Geometry check sheet. Reference: the model listing, model coordinates, mm. Face numbers are marked on the shaded views. A direction names the side the tool comes from. Give positions to 0.01 mm unless a question says otherwise; leave off trailing zeros. Loops run counter-clockwise (first coordinate to the right, second up) from the corner with the lowest first, then second, coordinate; pieces in that order, holes last. Notation, with made-up numbers: (65.25, 68.25) -> (124.25, 68.25) arc R19 ccw to (124.25, 85.25) -> close; hole circle Ø1 at (41, -15). An arc over 180 degrees is marked (long way). Answer as a JSON object with one key per item and string values.
from build123d import *

# Parameters (mm, degrees)
CHAMFER_1_SIZE           = 1
FILLET_1_R               = 2
CUT_EXTRUDE_1_DEPTH      = 99.642029582
CUT_EXTRUDE_1_DEPTH_BACK = 99.642029582
SKETCH_3_R               = 2.5


with BuildPart() as part:
    # 草图1 → 旋转1 (revolve)
    with BuildSketch(Plane.XY, mode=Mode.PRIVATE) as revolve_1_sk:
        with BuildLine():
            Line((0, 14.5), (13.774977314, 14.5))
            ThreePointArc((13.774977314, 14.5), (19.953843795, 1.357982993), (15.612494996, -12.5))
            Line((15.612494996, -12.5), (10.5, -12.5))
            Line((10.5, -12.5), (14.7, -39.5))
            Line((14.7, -39.5), (13.4, -69.5))
            Line((13.4, -69.5), (11.5, -69.5))
            Line((11.5, -69.5), (11.5, -94.5))
            Line((11.5, -94.5), (0, -94.5))
            Line((0, -94.5), (0, -12.5))
            Line((0, -12.5), (0, 14.5))
        make_face()
    revolve(revolve_1_sk.sketch.rotate(Axis((0, 41.043678396, 0), (0, -1, 0)), 90), axis=Axis((0, 41.043678396, 0), (0, -1, 0)))

    # 倒角1
    chamfer_1_edges = [part.edges().sort_by_distance(p)[0] for p in [
        (0, -94.5, -11.5),
    ]]
    chamfer(chamfer_1_edges, length=CHAMFER_1_SIZE)

    # 圆角1
    fillet_1_edges = [part.edges().sort_by_distance(p)[0] for p in [
        (0, -12.5, -10.5),
    ]]
    fillet(fillet_1_edges, radius=FILLET_1_R)

    # 草图3 → 切除-拉伸1 (cut, two sides: drawn at the far end of the back side and taken through both)
    with BuildSketch(Plane.XY.offset(-CUT_EXTRUDE_1_DEPTH_BACK)):
        with Locations((0, -88.5)):
            Circle(SKETCH_3_R)
    extrude(amount=CUT_EXTRUDE_1_DEPTH + CUT_EXTRUDE_1_DEPTH_BACK, mode=Mode.SUBTRACT)


solid = part.part
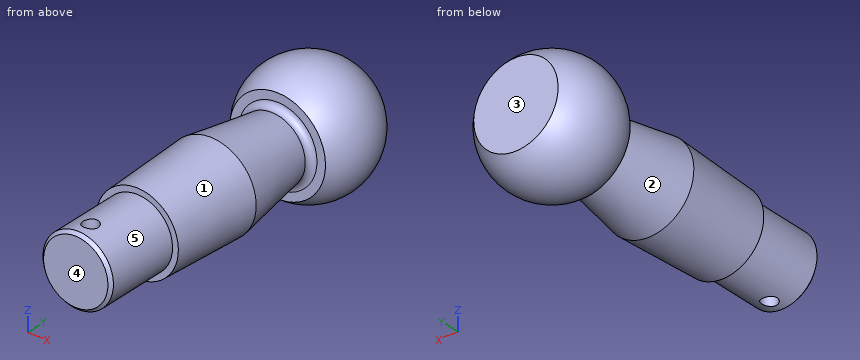
1) Section check B-B on z = 0. Record the cut outline in (x, y), plus the area to 3 significant figures.
Geometry check:
{"outline": "(-15.61, -12.5) -> (-12.84, -12.5) arc R2 cw to (-10.86, -14.81) -> (-14.7, -39.5) -> (-13.4, -69.5) -> (-11.5, -69.5) -> (-11.5, -93.5) -> (-10.5, -94.5) -> (10.5, -94.5) -> (11.5, -93.5) -> (11.5, -69.5) -> (13.4, -69.5) -> (14.7, -39.5) -> (10.86, -14.81) arc R2 cw to (12.84, -12.5) -> (15.61, -12.5) arc R20 ccw to (13.77, 14.5) -> (-13.77, 14.5) arc R20 ccw to start; hole circle Ø5 at (0, -88.5)", "area": "3,070 mm2"}
2) Tool access check on the marked faces 4 and 5. Record the directions out of +Z, -Z, +X, -X, +Y, -Y that give a thin tool (end or side, any length) a straight path to the whole face; none if there is none.
Geometry check:
{"face 4": "+Z, -Z, +X, -X, -Y", "face 5": "-Y"}
3) Section check A-A on x = 0. Record the cut outline in (y, z), plus the area to 3 significant figures.
Geometry check:
{"outline": "(-94.5, -10.5) -> (-93.5, -11.5) -> (-91, -11.5) -> (-91, 11.5) -> (-93.5, 11.5) -> (-94.5, 10.5) -> close; (-86, -11.5) -> (-69.5, -11.5) -> (-69.5, -13.4) -> (-39.5, -14.7) -> (-14.81, -10.86) arc R2 cw to (-12.5, -12.84) -> (-12.5, -15.61) arc R20 ccw to (14.5, -13.77) -> (14.5, 13.77) arc R20 ccw to (-12.5, 15.61) -> (-12.5, 12.84) arc R2 cw to (-14.81, 10.86) -> (-39.5, 14.7) -> (-69.5, 13.4) -> (-69.5, 11.5) -> (-86, 11.5) -> close", "area": "2,970 mm2"}
4) Draft check along Y on the marked faces 1, 2 and 3. Enter one of: pulls with the +Y half, pulls with the -Y half, needs draft (parallel to the pull), parting line crosses it, or undercut.
Geometry check:
{"face 1": "pulls with the -Y half", "face 2": "undercut", "face 3": "pulls with the +Y half"}
5) Section check D-D on y = 7. Record the cut outline in (x, z) (3 decimals), plus the area to 3 significant figures.
Geometry check:
{"outline": "circle Ø37.47 at (0, 0)", "area": "1,100 mm2"}
6) Section check C-C on y = -88.5. Record the cut outline in (x, z), plus the area to 3 significant figures.
Geometry check:
{"outline": "(-2.5, -11.22) -> (-2.5, 11.22) arc R11.5 ccw to start; (2.5, -11.22) arc R11.5 ccw to (2.5, 11.22) -> close", "area": "301 mm2"}
7) Depth check by flat-ended pin: P1, Ø6.5, axis at x = 0, y = -88.5, coming from the -Z side; P2, Ø6, axis at y = -77, z = -15.5, coming from the -X side; P3, Ø1, axis at y = -40, z = -5.5, coming from the +X side; P4, Ø5, axis at x = 8.5, y = -28, coming from the +Z side. Enter the tip coordinate at first touch or a pass-through.
Geometry check:
{"P1": "stops at z = -11.5", "P2": "passes through", "P3": "stops at x = 13.8", "P4": "stops at z = 11.5"}
8) Material ranges on line 1 along Y through (x, z) = (0, 2); line 2 along X through (y, z) = (-72, 0.5); line 3 along X through (y, z) = (-88.5, 2), recorded low to high. Write a range as from..to.
Geometry check:
{"line 1": "y = -94.5..-91, -86..14.5", "line 2": "x = -11.49..11.49", "line 3": "x = -11.32..-2.5, 2.5..11.32"}
